Geometry check sheet. Reference: the model listing, model coordinates, mm. Face numbers are marked on the shaded views. A direction names the side the tool comes from. Give positions to 0.01 mm unless a question says otherwise; leave off trailing zeros. Write each loop counter-clockwise with the first axis right and the second up, starting at its lowest first coordinate (ties: lowest second). Pieces come first, ordered by that corner, then holes. Notation, with made-up numbers: (88.25, -35.5) - (118.25, -35.5) arc R9 ccw to (118.25, -25.5) - close; hole circle Ø9 at (43.25, 26.25). An arc over 180 degrees is marked (long way). Write item = value, one per line. Start each with the question number.
(1) Draft check along X on the marked faces 3, 4 and 5. Enter one of: pulls with the +X half, pulls with the -X half, needs draft (parallel to the pull), parting line crosses it, or undercut.
(2) Thickness scan on L1, parallel to X at y = 5.85, z = 0; L2, parallel to X at y = 8.85, z = 0; L3, parallel to X at y = 9.25, z = -3. Record the ranges inside material, lowest first.
(3) Access from +Z, -Z, +X, -X, +Y, -Y to the whole of each face (thin tool, end or side, straight path). Record for the marked faces 1 and 2.
(4) Section check B-B, the plane y = 0. Enter the section's corners in (x, z), plus the area to 3 significant figures.
(5) Section check C-C, the plane x = 10.75. Enter the section's corners in (y, z).
(6) Section check A-A, the plane z = 0. Enter the section's corners in (x, y), plus the area to 3 significant figures.
(7) Section check D-D, the plane y = 7.5. Enter the section's corners in (x, z), plus the area to 3 significant figures.
(8) Depth check by flat-ended pin: pin 1 Ø3 at (y, z) = (-2.5, 1) entering from -X; pin 2 Ø1.5 at (x, z) = (2, -2.5) entering from +Y; pin 3 Ø1 at (x, z) = (2.5, -4) entering from -Y. Enter the tip coordinate at first touch or a pass-through.
```python
from build123d import *

# Parameters (mm, degrees)
SKETCH2_OUTSIDE_W      = 28.144
SKETCH2_OUTSIDE_H      = 28.144
SKETCH2_OUTSIDE_W_2    = 18
SKETCH2_OUTSIDE_H_2    = 25
CUT_EXTRUDE1_DEPTH     = 19.547236991
M4_TAPPED_HOLE1_REACH  = 27
M4_TAPPED_HOLE1_BORE_R = 1.65


with BuildPart() as part:
    # Sketch1 → Revolve1 (revolve)
    with BuildSketch(Plane.XY, mode=Mode.PRIVATE) as revolve1_sk:
        Polygon((0, 5), (0, 10), (11, 10), (11, 8), (12, 8), (12, 5), align=None)
    revolve(revolve1_sk.sketch.rotate(Axis((0, 0, 0), (1, 0, 0)), 90), axis=Axis((0, 0, 0), (1, 0, 0)))

    # Sketch2 outside → Cut-Extrude1 (cut, through all)
    with BuildSketch(Plane.ZY):
        Rectangle(SKETCH2_OUTSIDE_W, SKETCH2_OUTSIDE_H)
        Rectangle(SKETCH2_OUTSIDE_W_2, SKETCH2_OUTSIDE_H_2, mode=Mode.SUBTRACT)
    extrude(amount=-CUT_EXTRUDE1_DEPTH, mode=Mode.SUBTRACT)

    # M4 Tapped Hole1 bore → M4 Tapped Hole1 (cut, up to next)
    with BuildSketch(Plane(origin=(0, 10, 0), x_dir=(-1, 0, 0), z_dir=(0, 1, 0)), mode=Mode.PRIVATE) as m4_tapped_hole1_sk1:
        with Locations((-6, 0)):
            Circle(M4_TAPPED_HOLE1_BORE_R)
    m4_tapped_hole1_tool1 = extrude(m4_tapped_hole1_sk1.sketch, amount=-M4_TAPPED_HOLE1_REACH, mode=Mode.PRIVATE) & part.part
    add(m4_tapped_hole1_tool1.solids().sort_by_distance((6, 10, 0))[0], mode=Mode.SUBTRACT)


solid = part.part
```
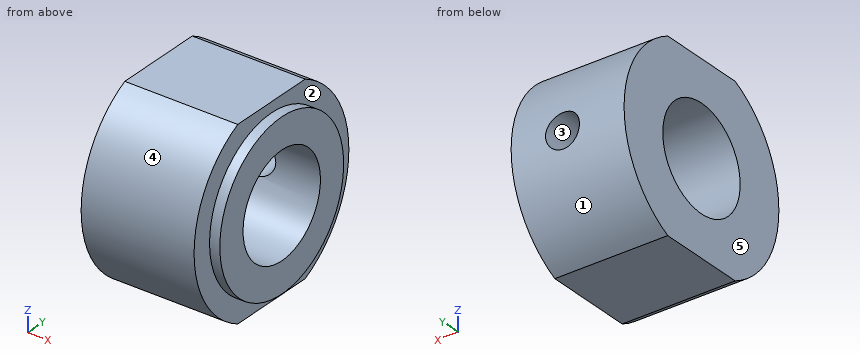
Model answer:
q1.face_3 = undercut
q1.face_4 = needs draft
q1.face_5 = pulls with the -X half
q2.L1 = 0 to 4.35, 7.65 to 12
q2.L2 = 0 to 4.35, 7.65 to 11
q2.L3 = 0 to 11
q3.face_1 = +X, -X, +Y
q3.face_2 = +X
q4.outline = (0, -9) - (11, -9) - (11, -8) - (12, -8) - (12, -5) - (0, -5) - close; (0, 5) - (12, 5) - (12, 8) - (11, 8) - (11, 9) - (0, 9) - close
q4.area = 94.0 mm²
q5.outline = (-4.36, -9) - (4.36, -9) arc R10 ccw to (4.36, 9) - (-4.36, 9) arc R10 ccw to start; hole circle Ø10 at (0, 0)
q6.outline = (0, -10) - (11, -10) - (11, -8) - (12, -8) - (12, -5) - (0, -5) - close; (0, 5) - (4.35, 5) - (4.35, 10) - (0, 10) - close; (7.65, 5) - (12, 5) - (12, 8) - (11, 8) - (11, 10) - (7.65, 10) - close
q6.area = 99.5 mm²
q7.outline = (0, -6.61) - (11, -6.61) - (11, -2.78) - (12, -2.78) - (12, 2.78) - (11, 2.78) - (11, 6.61) - (0, 6.61) - close; hole circle Ø3.3 at (6, 0)
q7.area = 143 mm²
q8.pin_1 = through
q8.pin_2 = 9.85
q8.pin_3 = -9.37
